Can you work these out from the model? Positions are in its coordinate system, mm. A direction names the side the tool comes from. Round coordinates to 2 decimals unless told otherwise and drop trailing zeros. Order: outer loops, then holes, each group sorted by start corner. A loop starts at its lowest first (then second) coordinate and runs counter-clockwise, first axis right, second up. Notation, with made-up numbers: (-8, -22.75) -> (3, -22.75) arc R17 ccw to (3, -9.75) -> close; hole circle Ø3 at (-19, -36). An arc over 180 degrees is marked (long way). Use a Markdown table: item, result. Add a question column.
Q1. If we section it at A-A on z = 68.5: List the corners of the cut face in (x, y) for me.
Q2. If we section it at B-B on y = -32.5: List the corners of the cut face in (x, z) for me.
Q3. If we section it at D-D on y = 28: List the corners of the cut face in (x, z) for me, plus the area to 3 significant figures.
Q4. I'm going to push a flat-ended pin straight in: pin 1 Ø8 at (y, z) = (-32.5, -87.5) entering from +X. Where does the tip first touch, or does it pass through?
Q5. If we section it at C-C on z = -87.5: List the corners of the cut face in (x, y) for me.
Q6. I need wall thicknesses on line 1 along Y through (x, z) = (11.8, -87.5); line 2 along Y through (x, z) = (4, 68.5); line 3 along Z through (x, y) = (3.25, 29.5). Which ranges of each line are inside material? Lowest first, please. Write a range as [from, to].
Q7. For faces 1 (the face through (3.549, 5.794, -7.161)), 2 (the face through (7, 5, -8)), which set-ups out of +Z, -Z, +X, -X, +Y, -Y let a thin tool reach every point of the face, with its end or its side?
Q8. We'd pull the mould along Y, two halves only. Please class faces 3 (the face through (3.5, 28.1, -84.5)), 4 (the face through (6, 40, 1)), 5 (the face through (6, -40, 1)), 6 (the face through (3.55, -31.6, -12.36)): +Y half, -Y half, draft (parallel to the pull), parting line (faces both ways), or undercut.
```python
from build123d import *

# Parameters (mm, degrees)
SKETCH1_W           = 188
SKETCH1_H           = 80
BOSS_EXTRUDE1_DEPTH = 13
SKETCH3_R           = 5
SKETCH3_R_2         = 3
CUT_EXTRUDE1_DEPTH  = 6
CUT_EXTRUDE2_REACH  = 104.981
SKETCH3_3_R         = 3
SKETCH4_R           = 5
SKETCH4_R_2         = 3
CUT_EXTRUDE3_DEPTH  = 6
CUT_EXTRUDE4_REACH  = 104.981
SKETCH4_3_R         = 3
SKETCH5_R           = 5
SKETCH5_R_2         = 3
CUT_EXTRUDE5_DEPTH  = 6
CUT_EXTRUDE6_REACH  = 104.981
SKETCH5_3_R         = 3


with BuildPart() as part:
    # Sketch1 → Boss-Extrude1 (new body)
    with BuildSketch(Plane(origin=(0, 0, 0), x_dir=(0, 0, -1), z_dir=(1, 0, 0))):
        Rectangle(SKETCH1_W, SKETCH1_H)
    extrude(amount=BOSS_EXTRUDE1_DEPTH)

    # Sketch3 → Cut-Extrude1 (cut)
    with BuildSketch(Plane(origin=(13, 0, 0), x_dir=(0, 0, -1), z_dir=(1, 0, 0))):
        with Locations((4.3, 4.893325501)):
            Circle(SKETCH3_R)
        with Locations((4.3, 4.893325501)):
            Circle(SKETCH3_R_2, mode=Mode.SUBTRACT)
    extrude(amount=-CUT_EXTRUDE1_DEPTH, mode=Mode.SUBTRACT)

    # Sketch3<3> → Cut-Extrude2 (cut, up to next)
    with BuildSketch(Plane(origin=(13, 0, 0), x_dir=(0, 0, -1), z_dir=(1, 0, 0)), mode=Mode.PRIVATE) as cut_extrude2_sk1:
        with Locations((4.3, 4.893325501)):
            Circle(SKETCH3_3_R)
    cut_extrude2_tool1 = extrude(cut_extrude2_sk1.sketch, amount=-CUT_EXTRUDE2_REACH, mode=Mode.PRIVATE) & part.part
    add(cut_extrude2_tool1.solids().sort_by_distance((13, 4.893326, -4.3))[0], mode=Mode.SUBTRACT)

    # Sketch4 → Cut-Extrude3 (cut)
    # profile 1 of 3: a face of its own
    with BuildSketch(Plane(origin=(13, 0, 0), x_dir=(0, 0, -1), z_dir=(1, 0, 0))):
        with Locations((-68.5, -32.5)):
            Circle(SKETCH4_R)
        with Locations((-68.5, -32.5)):
            Circle(SKETCH4_R_2, mode=Mode.SUBTRACT)
    # profile 2 of 3: a face of its own
    with BuildSketch(Plane(origin=(13, 0, 0), x_dir=(0, 0, -1), z_dir=(1, 0, 0))):
        with Locations((9.5, -32.5)):
            Circle(SKETCH4_R)
        with Locations((9.5, -32.5)):
            Circle(SKETCH4_R_2, mode=Mode.SUBTRACT)
    # profile 3 of 3: a face of its own
    with BuildSketch(Plane(origin=(13, 0, 0), x_dir=(0, 0, -1), z_dir=(1, 0, 0))):
        with Locations((87.5, -32.5)):
            Circle(SKETCH4_R)
        with Locations((87.5, -32.5)):
            Circle(SKETCH4_R_2, mode=Mode.SUBTRACT)
    extrude(amount=-CUT_EXTRUDE3_DEPTH, mode=Mode.SUBTRACT)

    # Sketch4<3> → Cut-Extrude4 (cut, up to next)
    with BuildSketch(Plane(origin=(13, 0, 0), x_dir=(0, 0, -1), z_dir=(1, 0, 0)), mode=Mode.PRIVATE) as cut_extrude4_sk1:
        with Locations((-68.5, -32.5)):
            Circle(SKETCH4_3_R)
    cut_extrude4_tool1 = extrude(cut_extrude4_sk1.sketch, amount=-CUT_EXTRUDE4_REACH, mode=Mode.PRIVATE) & part.part
    # Sketch4<3> → Cut-Extrude4 (cut, up to next)
    with BuildSketch(Plane(origin=(13, 0, 0), x_dir=(0, 0, -1), z_dir=(1, 0, 0)), mode=Mode.PRIVATE) as cut_extrude4_sk2:
        with Locations((9.5, -32.5)):
            Circle(SKETCH4_3_R)
    cut_extrude4_tool2 = extrude(cut_extrude4_sk2.sketch, amount=-CUT_EXTRUDE4_REACH, mode=Mode.PRIVATE) & part.part
    # Sketch4<3> → Cut-Extrude4 (cut, up to next)
    with BuildSketch(Plane(origin=(13, 0, 0), x_dir=(0, 0, -1), z_dir=(1, 0, 0)), mode=Mode.PRIVATE) as cut_extrude4_sk3:
        with Locations((87.5, -32.5)):
            Circle(SKETCH4_3_R)
    cut_extrude4_tool3 = extrude(cut_extrude4_sk3.sketch, amount=-CUT_EXTRUDE4_REACH, mode=Mode.PRIVATE) & part.part
    add(cut_extrude4_tool1.solids().sort_by_distance((13, -32.5, 68.5))[0], mode=Mode.SUBTRACT)
    add(cut_extrude4_tool2.solids().sort_by_distance((13, -32.5, -9.5))[0], mode=Mode.SUBTRACT)
    add(cut_extrude4_tool3.solids().sort_by_distance((13, -32.5, -87.5))[0], mode=Mode.SUBTRACT)

    # Sketch5 → Cut-Extrude5 (cut)
    with BuildSketch(Plane(origin=(13, 0, 0), x_dir=(0, 0, -1), z_dir=(1, 0, 0))):
        with Locations((87.5, 28)):
            Circle(SKETCH5_R)
        with Locations((87.5, 28)):
            Circle(SKETCH5_R_2, mode=Mode.SUBTRACT)
    extrude(amount=-CUT_EXTRUDE5_DEPTH, mode=Mode.SUBTRACT)

    # Sketch5<3> → Cut-Extrude6 (cut, up to next)
    with BuildSketch(Plane(origin=(13, 0, 0), x_dir=(0, 0, -1), z_dir=(1, 0, 0)), mode=Mode.PRIVATE) as cut_extrude6_sk1:
        with Locations((87.5, 28)):
            Circle(SKETCH5_3_R)
    cut_extrude6_tool1 = extrude(cut_extrude6_sk1.sketch, amount=-CUT_EXTRUDE6_REACH, mode=Mode.PRIVATE) & part.part
    add(cut_extrude6_tool1.solids().sort_by_distance((13, 28, -87.5))[0], mode=Mode.SUBTRACT)


solid = part.part
```
Answer below:
| question | item | result |
|---|---|---|
| 1 | outline | (0, -40) -> (13, -40) -> (13, -37.5) -> (7, -37.5) -> (7, -35.5) -> (0, -35.5) -> close; (0, -29.5) -> (7, -29.5) -> (7, -27.5) -> (13, -27.5) -> (13, 40) -> (0, 40) -> close |
| 2 | outline | (0, -94) -> (13, -94) -> (13, -92.5) -> (7, -92.5) -> (7, -90.5) -> (0, -90.5) -> close; (0, -84.5) -> (7, -84.5) -> (7, -82.5) -> (13, -82.5) -> (13, -14.5) -> (7, -14.5) -> (7, -12.5) -> (0, -12.5) -> close; (0, -6.5) -> (7, -6.5) -> (7, -4.5) -> (13, -4.5) -> (13, 63.5) -> (7, 63.5) -> (7, 65.5) -> (0, 65.5) -> close; (0, 71.5) -> (7, 71.5) -> (7, 73.5) -> (13, 73.5) -> (13, 94) -> (0, 94) -> close |
| 3 | outline | (0, -94) -> (13, -94) -> (13, -92.5) -> (7, -92.5) -> (7, -90.5) -> (0, -90.5) -> close; (0, -84.5) -> (7, -84.5) -> (7, -82.5) -> (13, -82.5) -> (13, 94) -> (0, 94) -> close |
| 3 | area | 2,340 mm² |
| 4 | pin 1 | x = 7 |
| 5 | outline | (0, -40) -> (13, -40) -> (13, -37.5) -> (7, -37.5) -> (7, -35.5) -> (0, -35.5) -> close; (0, -29.5) -> (7, -29.5) -> (7, -27.5) -> (13, -27.5) -> (13, 23) -> (7, 23) -> (7, 25) -> (0, 25) -> close; (0, 31) -> (7, 31) -> (7, 33) -> (13, 33) -> (13, 40) -> (0, 40) -> close |
| 6 | line 1 | [-40, -37.5], [-27.5, 23], [33, 40] |
| 6 | line 2 | [-40, -35.5], [-29.5, 40] |
| 6 | line 3 | [-94, -90.1], [-84.9, 94] |
| 7 | face 1 | +X, -X |
| 7 | face 2 | +X |
| 8 | face 3 | undercut |
| 8 | face 4 | +Y half |
| 8 | face 5 | -Y half |
| 8 | face 6 | undercut |
